```python
from build123d import *

# Parameters (mm, degrees)
M2_5_TAPPED_HOLE1_D     = 2.05
M2_5_TAPPED_HOLE1_DEPTH = 4.35
M2_5_TAPPED_HOLE1_TIP   = 0.615882135
SKETCH5_R               = 0.4
BOSS_EXTRUDE1_DEPTH     = 15
SKETCH6_R               = 4.15
CUT_EXTRUDE2_DEPTH      = 15


with BuildPart() as part:
    # Sketch1 → Revolve1 (revolve)
    with BuildSketch(Plane.XY, mode=Mode.PRIVATE) as revolve1_sk:
        with BuildLine():
            Line((1.625, 11.8), (9.45, 11.8))
            Line((9.45, 11.8), (9.45, 1))
            ThreePointArc((9.45, 1), (9.157106781, 0.292893219), (8.45, 0))
            Line((8.45, 0), (4.15, 0))
            Line((4.15, 0), (4.15, 6.3))
            Line((4.15, 6.3), (1.625, 6.3))
            Line((1.625, 6.3), (1.625, 11.8))
        make_face()
    revolve(revolve1_sk.sketch.rotate(Axis((0, 0, 0), (0, 1, 0)), 90), axis=Axis((0, 0, 0), (0, 1, 0)))

    # M2.5 Tapped Hole1
    with Locations(Plane(origin=(0, 11.8, 0), x_dir=(-1, 0, 0), z_dir=(0, 1, 0))):
        with Locations((0, -6.25), (0, 6.25)):
            Hole(M2_5_TAPPED_HOLE1_D / 2, depth=M2_5_TAPPED_HOLE1_DEPTH)
            with Locations((0, 0, -(M2_5_TAPPED_HOLE1_DEPTH + M2_5_TAPPED_HOLE1_TIP / 2))):  # 118° drill point
                Cone(0, M2_5_TAPPED_HOLE1_D / 2, M2_5_TAPPED_HOLE1_TIP, mode=Mode.SUBTRACT)

    # Sketch5 → Boss-Extrude1 (add)
    with BuildSketch(Plane.XY):
        with Locations(Location((-0.8, 1.2, 0), (0, 0, 180))):
            Circle(SKETCH5_R)
        with Locations(Location((0.7, 1.2, 0), (0, 0, 180))):
            Circle(SKETCH5_R)
    extrude(amount=BOSS_EXTRUDE1_DEPTH)

    # Sketch6 → Cut-Extrude2 (cut)
    with BuildSketch(Plane.XZ.offset(-6.3)):
        with Locations(Location((0, 0, 0), (0, 0, 270))):
            Circle(SKETCH6_R)
    extrude(amount=CUT_EXTRUDE2_DEPTH, mode=Mode.SUBTRACT)


solid = part.part
```
Input: part model. Units: mm. Frame: model coordinates. A direction names the side the tool comes from. Give positions to 0.01 mm unless a question says otherwise; leave off trailing zeros. Write each loop counter-clockwise with the first axis right and the second up, starting at its lowest first coordinate (ties: lowest second). Pieces come first, ordered by that corner, then holes. Notation, with made-up numbers: (-11, 21) - (32, 21) arc R30 cw to (32, 48) - close; hole circle Ø8 at (47.5, 40.25). An arc over 180 degrees is marked (long way). Write item = value, one per line. Start each with the question number.
1) Cut plane D-D (z = 11.25). Return loops of the section in (x, y).
2) Cut plane C-C (y = 5.75). Return loops of the section in (x, z).
3) Pin query (flat end, axial travel): pin 1 (2 mm diameter, centred on x = 7, y = 8.5, fed in from -Z); pin 2 (6.5 mm diameter, centred on x = 0, z = 0, fed in from -Y); pin 3 (4 mm diameter, centred on y = 8, z = -3.5, fed in from +X). Return the tip coordinate at first contact, or that it passes through.
4) Draft query along Z for faces 1 (the face through (2, 0, 4)), 2 (the face through (-0.22, 9.59, -7.25)), 3 (the face through (0.7, 1.2, 15)). Return one class per face: pulls with the +Z half, pulls with the -Z half, needs draft (parallel to the pull), parting line crosses it, or undercut.
5) Cut plane B-B (y = 9.5). Return loops of the section in (x, z) (3 decimals), and give its area (3 significant figures).
6) Cut plane A-A (z = 0). Return loops of the section in (x, y) (3 decimals), and give its area (3 significant figures).
7) Reachability of faces 4 (the face through (2, 6.3, 0)), 5 (the face through (-0.22, 9.59, 5.25)), 6 (the face through (0.995, 0.93, 12.154)) from +Z, -Z, +X, -X, +Y, -Y: full face, straight path, thin tool, end or side. Return the list, or none.
8) Material intervals for L1, parallel to X at y = 5, z = 0; L2, parallel to X at y = 10, z = 0 (3 decimals); L3, parallel to Z at x = -2.75, y = 4.25, sorted ascending. Write a range as [from, to].
Answers follow:
q1.outline = circle Ø0.8 at (-0.8, 1.2); circle Ø0.8 at (0.7, 1.2)
q2.outline = circle Ø18.9 at (0, 0); hole circle Ø8.3 at (0, 0)
q3.pin_1 = -7.3
q3.pin_2 = 6.3
q3.pin_3 = 9.33
q4.face_1 = needs draft
q4.face_2 = undercut
q4.face_3 = pulls with the +Z half
q5.outline = circle Ø18.9 at (0, 0); hole circle Ø3.25 at (0, 0); hole circle Ø2.05 at (0, -6.25); hole circle Ø2.05 at (0, 6.25)
q5.area = 266 mm^2
q6.outline = (-9.45, 1) arc R1 ccw to (-8.45, 0) - (-4.15, 0) - (-4.15, 6.3) - (-1.625, 6.3) - (-1.625, 11.8) - (-9.45, 11.8) - close; (1.625, 6.3) - (4.15, 6.3) - (4.15, 0) - (8.45, 0) arc R1 ccw to (9.45, 1) - (9.45, 11.8) - (1.625, 11.8) - close
q6.area = 152 mm^2
q7.face_4 = -Y
q7.face_5 = +Y
q7.face_6 = +Z
q8.L1 = [-9.45, -4.15], [4.15, 9.45]
q8.L2 = [-9.45, -1.625], [1.625, 9.45]
q8.L3 = [-9.04, -3.11], [3.11, 9.04]
